Job drawing, mm, ordinate dimensions from the low corner. One solid piece. A direction names the side the tool comes from. Round coordinates to 2 decimals unless told otherwise and drop trailing zeros. Write each loop counter-clockwise with the first axis right and the second up, starting at its lowest first coordinate (ties: lowest second). Pieces come first, ordered by that corner, then holes.
1) Which spindle directions (+Z, -Z, +X, -X, +Y, -Y) get a long thin tool onto all of the face, cutting with end or side? Do the marked faces 4 and 5. Say none if no direction does.
2) Flat gauge pin, fed straight in: pin 1 (5 mm diameter, centred on x = 47, z = 25, fed in from -Y). Where does the tip first touch, or does it go through?
3) Saw through at A-A on z = 50. Write the cut outline in (x, y), and give its area (3 significant figures).
4) Pull direction Y, two halves, no side cores. Call the marked faces 1, 2 and 3: +Y half, -Y half, draft (parallel to the pull), parting line (faces both ways), or undercut.
5) Drill centre lines: L1, parallel to Z at x = 9, y = 42; L2, parallel to Y at x = 29.5, z = 83.5; L3, parallel to X at y = 26, z = 7. Where is each one in solid material? Low to high.
6) Saw through at C-C on y = 52.5. Write the cut outline in (x, z).
7) Saw through at D-D on z = 39.5. Write the cut outline in (x, y), and give its area (3 significant figures).
8) Saw through at B-B on y = 42. Write the cut outline in (x, z), and give its area (3 significant figures).
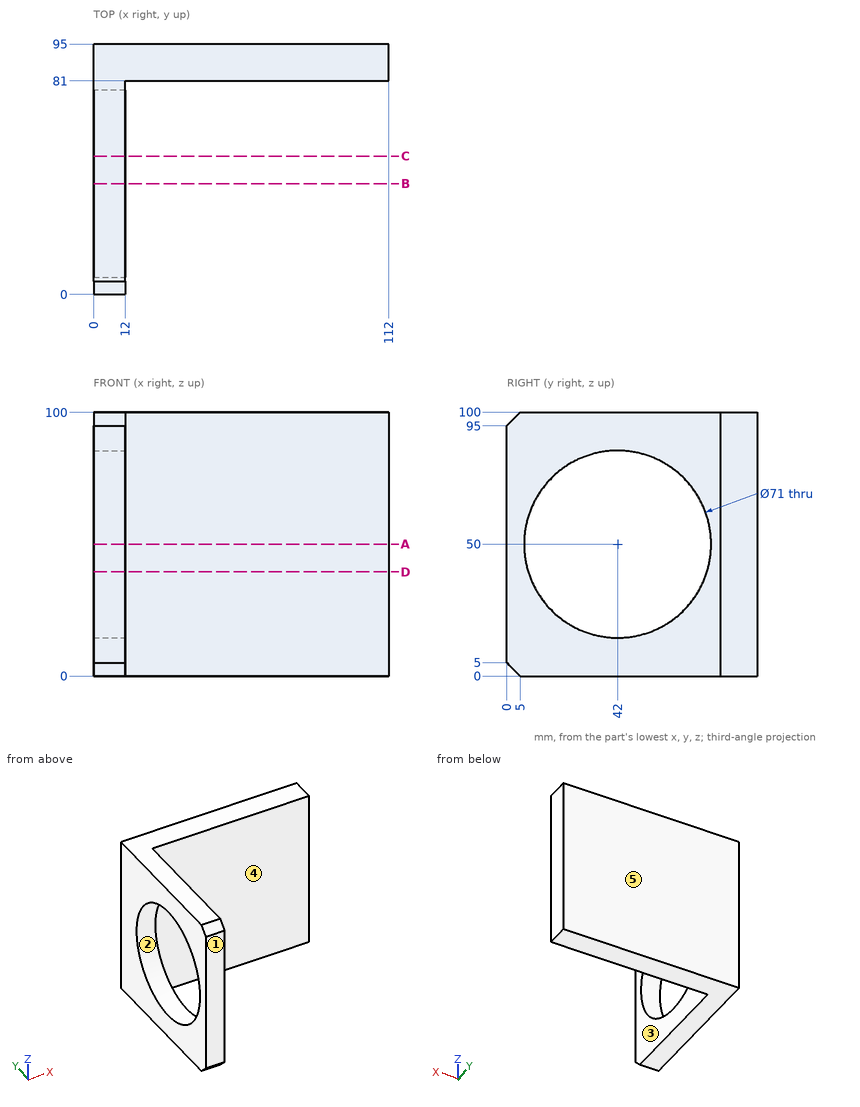
Completed:
1. face 4: +Z, -Z, +X, -Y
1. face 5: +Z, -Z, +X, -X, +Y
2. pin 1: stops at y = 81
3. outline: (0, 0) - (12, 0) - (12, 6.5) - (0, 6.5) - close; (0, 77.5) - (12, 77.5) - (12, 81) - (112, 81) - (112, 95) - (0, 95) - close
3. area: 1,690 mm2
4. face 1: -Y half
4. face 2: undercut
4. face 3: draft
5. L1: z = 0 to 14.5, 85.5 to 100
5. L2: y = 81 to 95
5. L3: x = 0 to 12
6. outline: (0, 0) - (12, 0) - (12, 16.09) - (0, 16.09) - close; (0, 83.91) - (12, 83.91) - (12, 100) - (0, 100) - close
7. outline: (0, 0) - (12, 0) - (12, 8.09) - (0, 8.09) - close; (0, 75.91) - (12, 75.91) - (12, 81) - (112, 81) - (112, 95) - (0, 95) - close
7. area: 1,730 mm2
8. outline: (0, 0) - (12, 0) - (12, 14.5) - (0, 14.5) - close; (0, 85.5) - (12, 85.5) - (12, 100) - (0, 100) - close
8. area: 348 mm2
